from build123d import *

# Parameters (mm, degrees)
BOSS_EXTRUDE1_DEPTH                                  = 15
CBORE_FOR_M5_HEXAGON_SOCKET_HEAD_CAP_SCR_D           = 5.5
CBORE_FOR_M5_HEXAGON_SOCKET_HEAD_CAP_SCR_CBORE_D     = 10
CBORE_FOR_M5_HEXAGON_SOCKET_HEAD_CAP_SCR_CBORE_DEPTH = 5.7
M5_CLEARANCE_HOLE1_D                                 = 5.5
CHAMFER1_SIZE                                        = 2


with BuildPart() as part:
    # Sketch1 → Boss-Extrude1 (new body)
    with BuildSketch(Plane(origin=(0, 0, 0), x_dir=(0, 0, -1), z_dir=(1, 0, 0))):
        Polygon((0, 0), (25, 0), (25, 12), (12, 12), (12, 221.5), (0, 221.5), align=None)
    extrude(amount=BOSS_EXTRUDE1_DEPTH)

    # CBORE for M5 Hexagon socket head cap screws1 (through all)
    with Locations(Plane(origin=(0, 0, -12), x_dir=(-1, 0, 0), z_dir=(0, 0, -1))):
        with Locations((-7.5, 45), (-7.5, 190)):
            CounterBoreHole(CBORE_FOR_M5_HEXAGON_SOCKET_HEAD_CAP_SCR_D / 2, CBORE_FOR_M5_HEXAGON_SOCKET_HEAD_CAP_SCR_CBORE_D / 2, CBORE_FOR_M5_HEXAGON_SOCKET_HEAD_CAP_SCR_CBORE_DEPTH)

    # M5 Clearance Hole1 (through all)
    with Locations(Plane(origin=(0, 0, 0), x_dir=(-1, 0, 0), z_dir=(0, -1, 0))):
        with Locations((-7.5, 18)):
            Hole(M5_CLEARANCE_HOLE1_D / 2)

    # Chamfer1
    chamfer1_edges = [part.edges().sort_by_distance(p)[0] for p in [
        (15, 6, -25),
        (15, 221.5, -6),
        (0, 221.5, -6),
        (0, 6, -25),
    ]]
    chamfer(chamfer1_edges, length=CHAMFER1_SIZE)


solid = part.part
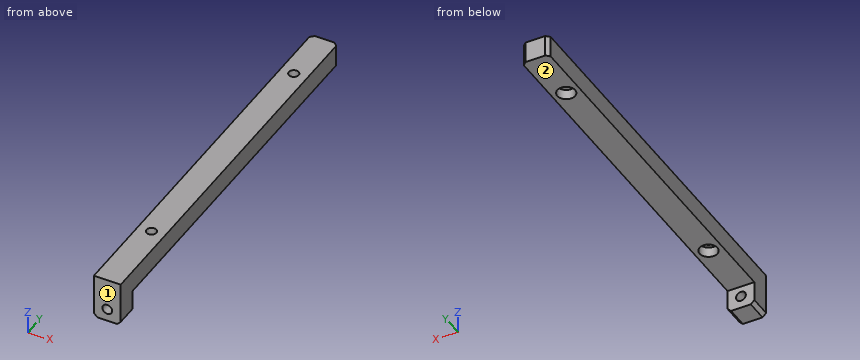
CAD build for the part. Positions are in the model's coordinates, mm. Face numbers are marked on the shaded views. A direction names the side the tool comes from. Coordinates: 2 decimals unless noted, no trailing zeros. Write each loop counter-clockwise with the first axis right and the second up, starting at its lowest first coordinate (ties: lowest second). Pieces come first, ordered by that corner, then holes. Notation, with made-up numbers: (30.25, 33.25) - (55.25, 33.25) arc R23 ccw to (55.25, 46.25) - close; hole circle Ø7 at (42, -31). An arc over 180 degrees is marked (long way). Use a Markdown table: item, result. Add a question column.
Item 1: 3-axis set-ups, long thin cutter, end or side, ignore diameter. For the marked faces 1 and 2: which of +Z, -Z, +X, -X, +Y, -Y reach the whole face in a straight line?
Item 2: Band-saw the part on B-B, the plane x = 7.5. Give the cut face in (y, z).
Item 3: Band-saw the part on D-D, the plane z = -18. Give the cut face in (x, y), and give its area (3 significant figures).
Item 4: Band-saw the part on C-C, the plane y = 190. Give the cut face in (x, z).
Item 5: Drill centre lines: L1, parallel to Y at x = 7.5, z = -8.2; L2, parallel to Y at x = 7.5, z = -5; L3, parallel to X at y = 9.5, z = -18. Where is each one in solid material? Low to high. Write a range as from..to.
Item 6: Flat gauge pins, fed straight in: pin 1 (4 mm diameter, centred on x = 4.5, z = -17, fed in from -Y); pin 2 (8 mm diameter, centred on x = 6.5, y = 188, fed in from -Z); pin 3 (3 mm diameter, centred on x = 7.5, z = -14.5, fed in from +Y); pin 4 (3 mm diameter, centred on x = 5, y = 47, fed in from -Z). Where does each tip first touch, or does it go through?
Item 7: Band-saw the part on A-A, the plane z = -3.5. Give the cut face in (x, y).
Numbers:
| question | item | result |
|---|---|---|
| 1 | face 1 | +Z, -Z, +X, -X, -Y |
| 1 | face 2 | -Z, +X, -X, +Y |
| 2 | outline | (0, -25) - (12, -25) - (12, -20.75) - (0, -20.75) - close; (0, -15.25) - (12, -15.25) - (12, -12) - (40, -12) - (40, -6.3) - (42.25, -6.3) - (42.25, 0) - (0, 0) - close; (47.75, -6.3) - (50, -6.3) - (50, -12) - (185, -12) - (185, -6.3) - (187.25, -6.3) - (187.25, 0) - (47.75, 0) - close; (192.75, -6.3) - (195, -6.3) - (195, -12) - (221.5, -12) - (221.5, 0) - (192.75, 0) - close |
| 3 | outline | (0, 0) - (4.75, 0) - (4.75, 12) - (0, 12) - close; (10.25, 0) - (15, 0) - (15, 12) - (10.25, 12) - close |
| 3 | area | 114 mm2 |
| 4 | outline | (0, -12) - (2.5, -12) - (2.5, -6.3) - (4.75, -6.3) - (4.75, 0) - (0, 0) - close; (10.25, -6.3) - (12.5, -6.3) - (12.5, -12) - (15, -12) - (15, 0) - (10.25, 0) - close |
| 5 | L1 | 0..40, 50..185, 195..221.5 |
| 5 | L2 | 0..42.25, 47.75..187.25, 192.75..221.5 |
| 5 | L3 | 0..4.75, 10.25..15 |
| 6 | pin 1 | y = 0 |
| 6 | pin 2 | z = -12 |
| 6 | pin 3 | y = 12 |
| 6 | pin 4 | z = -6.3 |
| 7 | outline | (0, 0) - (15, 0) - (15, 219.5) - (13, 221.5) - (2, 221.5) - (0, 219.5) - close; hole circle Ø5.5 at (7.5, 45); hole circle Ø5.5 at (7.5, 190) |
